```python
from build123d import *

# Parameters (mm, degrees)
BASE_BLOCK_PROFILE_W         = 850
BASE_BLOCK_PROFILE_H         = 225
BASE_BLOCK_850X225X106_DEPTH = 106
V_GROOVE_45DEG_DEPTH         = 864.939957404
T_SLOTS_2X_DEPTH             = 864.939957404
T_SLOT_END_POCKETS_REACH     = 454.236


with BuildPart() as part:
    # Base Block Profile → Base Block 850x225x106 (new body)
    with BuildSketch(Plane.XY):
        Rectangle(BASE_BLOCK_PROFILE_W, BASE_BLOCK_PROFILE_H)
    extrude(amount=BASE_BLOCK_850X225X106_DEPTH)

    # V-Groove Profile → V-Groove 45deg (cut, through all)
    with BuildSketch(Plane(origin=(425, 0, 0), x_dir=(0, 0, -1), z_dir=(1, 0, 0))):
        Polygon((-16, -112.5), (0, -112.5), (0, -100), (-16, -84), align=None)
        Polygon((-16, 84), (-16, 112.5), (0, 112.5), (0, 100), align=None)
    extrude(amount=-V_GROOVE_45DEG_DEPTH, mode=Mode.SUBTRACT)

    # T-Slots Profile → T-Slots 2x (cut, through all)
    with BuildSketch(Plane(origin=(425, 0, 0), x_dir=(0, 0, -1), z_dir=(1, 0, 0))):
        Polygon((-96, -12.5), (-84, -12.5), (-84, 12.5), (-96, 12.5), (-96, 8), (-106, 8), (-106, -8), (-96, -8), align=None)
        Polygon((-84, 77.5), (-84, 52.5), (-96, 52.5), (-96, 57), (-106, 57), (-106, 73), (-96, 73), (-96, 77.5), align=None)
        Polygon((-96, -77.5), (-84, -77.5), (-84, -52.5), (-96, -52.5), (-96, -57), (-106, -57), (-106, -73), (-96, -73), align=None)
    extrude(amount=-T_SLOTS_2X_DEPTH, mode=Mode.SUBTRACT)

    # T-Slot End Pockets: up to this face of the body (flat: up to its plane)
    t_slot_end_pockets_end = Plane(part.part.faces().sort_by_distance((0, 0, 84))[0])
    # T-Slot End Pockets Profile → T-Slot End Pockets (cut, up to the picked face)
    with BuildSketch(Plane.XY.offset(106), mode=Mode.PRIVATE) as t_slot_end_pockets_sk1:
        with BuildLine():
            Line((-399.363172475, -77.493249387), (-399.363172475, 77.493249387))
            ThreePointArc((-399.363172475, 77.493249387), (-380, 102.5), (-360.636827525, 77.493249387))
            Line((-360.636827525, 77.493249387), (-360.636827525, -77.493249387))
            ThreePointArc((-360.636827525, -77.493249387), (-380, -102.5), (-399.363172475, -77.493249387))
        make_face()
    t_slot_end_pockets_tool1 = split(extrude(t_slot_end_pockets_sk1.sketch, amount=-T_SLOT_END_POCKETS_REACH, mode=Mode.PRIVATE), bisect_by=t_slot_end_pockets_end, keep=Keep.BOTH, mode=Mode.PRIVATE)
    # T-Slot End Pockets Profile → T-Slot End Pockets (cut, up to the picked face)
    with BuildSketch(Plane.XY.offset(106), mode=Mode.PRIVATE) as t_slot_end_pockets_sk2:
        with BuildLine():
            Line((360.636827525, -77.493249387), (360.636827525, 77.493249387))
            ThreePointArc((360.636827525, 77.493249387), (380, 102.5), (399.363172475, 77.493249387))
            Line((399.363172475, 77.493249387), (399.363172475, -77.493249387))
            ThreePointArc((399.363172475, -77.493249387), (380, -102.5), (360.636827525, -77.493249387))
        make_face()
    t_slot_end_pockets_tool2 = split(extrude(t_slot_end_pockets_sk2.sketch, amount=-T_SLOT_END_POCKETS_REACH, mode=Mode.PRIVATE), bisect_by=t_slot_end_pockets_end, keep=Keep.BOTH, mode=Mode.PRIVATE)
    add(t_slot_end_pockets_tool1.solids().sort_by(Axis((-380, 0, 106), (0, 0, -1)))[0], mode=Mode.SUBTRACT)
    add(t_slot_end_pockets_tool2.solids().sort_by(Axis((380, 0, 106), (0, 0, -1)))[0], mode=Mode.SUBTRACT)


solid = part.part
```
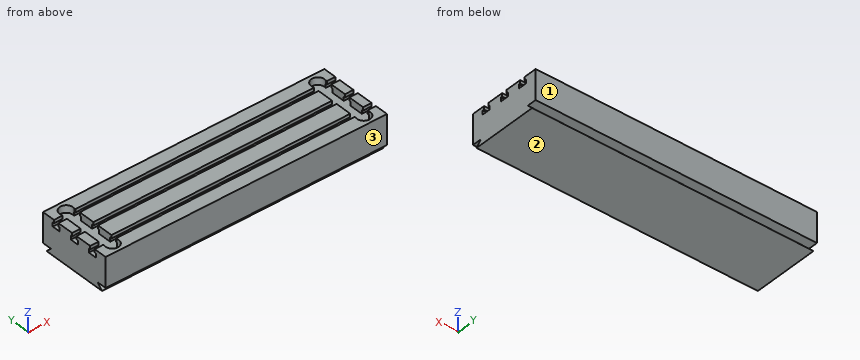
Check sheet for the modelled part. Datum: model origin and axes. Units: mm. Face numbers are marked on the shaded views. Round coordinates to 2 decimals unless told otherwise and drop trailing zeros. Order: outer loops, then holes, each group sorted by start corner. A loop starts at its lowest first (then second) coordinate and runs counter-clockwise, first axis right, second up. Notation, with made-up numbers: (73, 63) - (115, 63) arc R24 cw to (115, 93) - close; hole circle Ø2 at (88, 37). An arc over 180 degrees is marked (long way). Answer as CSV lines item,"result". Start each with the question number.
1) Draft check along Y on the marked faces 1, 2 and 3. Enter one of: +Y half, -Y half, draft (parallel to the pull), parting line (faces both ways), or undercut.
2) Scan lines: probe 1 along X at (y, z) = (-82.5, 96.5); probe 2 along Y at (x, z) = (289, 95); probe 3 along Y at (x, z) = (351, 99). Record each from-to range of solid material in increasing order.
3) Section check B-B (y = 22). Record the cut outline in (x, z), then the cut area to 3 significant figures.
4) Section check C-C (x = 380). Record the cut outline in (y, z).
5) Depth check by flat-ended pin: pin 1 (3.5 mm diameter, centred on x = 115.5, y = 54.5, fed in from -Z). Enter the tip coordinate at first touch or a pass-through.
Determined:
1,face 1,"+Y half"
1,face 2,"draft"
1,face 3,"-Y half"
2,probe 1,"-425 to -400, -360 to 360, 400 to 425"
2,probe 2,"-112.5 to -77.5, -52.5 to -12.5, 12.5 to 52.5, 77.5 to 112.5"
2,probe 3,"-112.5 to -73, -57 to -8, 8 to 57, 73 to 112.5"
3,outline,"(-425, 0) - (425, 0) - (425, 106) - (399.36, 106) - (399.36, 84) - (360.64, 84) - (360.64, 106) - (-360.64, 106) - (-360.64, 84) - (-399.36, 84) - (-399.36, 106) - (-425, 106) - close"
3,area,"88,400 mm^2"
4,outline,"(-112.5, 16) - (-84, 16) - (-100, 0) - (100, 0) - (84, 16) - (112.5, 16) - (112.5, 106) - (102.5, 106) - (102.5, 84) - (-102.5, 84) - (-102.5, 106) - (-112.5, 106) - close"
5,pin 1,"z = 0"
